Here's how the part is built. I have some questions about the finished solid (model axes, mm). Face numbers are marked on the shaded views. A direction names the side the tool comes from. Coordinates: 2 decimals unless noted, no trailing zeros. Write each loop counter-clockwise with the first axis right and the second up, starting at its lowest first coordinate (ties: lowest second). Pieces come first, ordered by that corner, then holes. Notation, with made-up numbers: (-17, 22) -> (42, 22) arc R29 ccw to (42, 57) -> close; hole circle Ø8 at (18.25, 87). An arc over 180 degrees is marked (long way). Use a Markdown table: item, result. Add a question column.
```python
from build123d import *

# Parameters (mm, degrees)
EXTRUDE1_DEPTH      = 7
EXTRUDE2_DEPTH      = 146.223964964
EXTRUDE2_DEPTH_BACK = 146.223964964
SKETCH2_R           = 2.6
SKETCH5_W           = 6
SKETCH5_H           = 3.7
EXTRUDE5_DEPTH      = 146.292807805
EXTRUDE6_DEPTH      = 3.7


with BuildPart() as part:
    # Sketch1 → Extrude1 (new, symmetric)
    with BuildSketch(Plane.XY):
        with BuildLine():
            Line((0, 0), (27.422252789, 0))
            ThreePointArc((27.422252789, 0), (27.989575353, 0.05413084), (28.536424818, 0.214569927))
            Line((28.536424818, 0.214569927), (37.105958636, 3.642383454))
            ThreePointArc((37.105958636, 3.642383454), (38.017374412, 3.909781934), (38.962912018, 4))
            Line((38.962912018, 4), (145, 4))
            Line((145, 4), (145, 2))
            Line((145, 2), (38.962912018, 2))
            ThreePointArc((38.962912018, 2), (38.395589454, 1.94586916), (37.848739989, 1.785430073))
            Line((37.848739989, 1.785430073), (29.279206171, -1.642383454))
            ThreePointArc((29.279206171, -1.642383454), (28.367790395, -1.909781934), (27.422252789, -2))
            Line((27.422252789, -2), (0, -2))
            Line((0, -2), (0, 0))
        make_face()
    extrude(amount=EXTRUDE1_DEPTH, both=True)

    # Sketch2 → Extrude2 (cut, two sides: drawn at the far end of the back side and taken through both)
    with BuildSketch(Plane(origin=(0, 0, 0), x_dir=(1, 0, 0), z_dir=(0, 1, 0)).offset(-EXTRUDE2_DEPTH_BACK)):
        with Locations(Location((8, 0, 0), (0, 0, 270))):
            Circle(SKETCH2_R)
        with Locations(Location((112, 0, 0), (0, 0, 270))):
            Circle(SKETCH2_R)
        with BuildLine():
            Line((138, 7), (138, 13.502314884))
            Line((138, 13.502314884), (156.33198023, 13.502314884))
            Line((156.33198023, 13.502314884), (156.33198023, -14.26269046))
            Line((156.33198023, -14.26269046), (138, -14.26269046))
            Line((138, -14.26269046), (138, -7))
            ThreePointArc((138, -7), (145, 0), (138, 7))
        make_face()
        with BuildLine():
            Line((7, 7), (7, 12.663603668))
            Line((7, 12.663603668), (-7.097085647, 12.663603668))
            Line((-7.097085647, 12.663603668), (-7.097085647, -11.053510543))
            Line((-7.097085647, -11.053510543), (7, -11.053510543))
            Line((7, -11.053510543), (7, -7))
            ThreePointArc((7, -7), (0, 0), (7, 7))
        make_face()
    extrude(amount=EXTRUDE2_DEPTH + EXTRUDE2_DEPTH_BACK, mode=Mode.SUBTRACT)

    # Sketch5 → Extrude5 (cut, through all)
    with BuildSketch(Plane(origin=(0, 4, 0), x_dir=(1, 0, 0), z_dir=(0, 1, 0))):
        with Locations((130, 5.15)):
            Rectangle(SKETCH5_W, SKETCH5_H)
    extrude(amount=-EXTRUDE5_DEPTH, mode=Mode.SUBTRACT)

    # Sketch6 → Extrude6 (add)
    with BuildSketch(Plane.XY.offset(-7)):
        with BuildLine():
            Line((125.978380641, 4), (124.313573726, 4))
            Line((124.313573726, 4), (124.313573726, 2))
            Line((124.313573726, 2), (126.730778484, 2))
            ThreePointArc((126.730778484, 2), (127.10118691, 2.071131011), (127.418900283, 2.274404804))
            ThreePointArc((127.418900283, 2.274404804), (129.995755169, 3.923082851), (133, 4.5))
            Line((133, 4.5), (133, 6.5))
            ThreePointArc((133, 6.5), (129.608718605, 5.914287154), (126.61035388, 4.22500979))
            ThreePointArc((126.61035388, 4.22500979), (126.313798135, 4.057930414), (125.978380641, 4))
        make_face()
    extrude(amount=EXTRUDE6_DEPTH)


solid = part.part
```
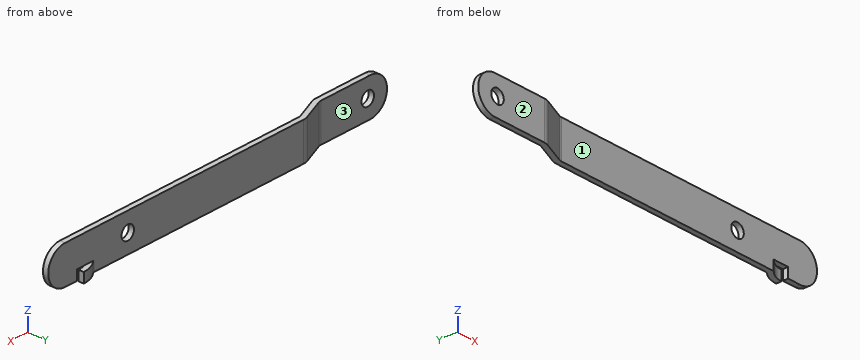
Q1. Suppose I cut it at D-D, the plane x = 80.5. Write out the boundary of the cut face in (y, z), and give its area (3 significant figures).
Q2. Suppose I cut it at C-C, the plane z = 5.5. Write out the boundary of the cut face in (x, y).
Q3. Suppose I cut it at B-B, the plane z = -0.5. Write out the boundary of the cut face in (x, y).
Q4. Will these pins go through, and if not, where does the flat tip stop? pin 1 (1 mm diameter, centred on y = 5.5, z = -5.5, fed in from +X); pin 2 (3 mm diameter, centred on y = 4.5, z = -5, fed in from +X); pin 3 (1.5 mm diameter, centred on y = -1, z = -2, fed in from -X).
Q5. Please list where these lines run through material, in increasing order: line 1 (Z direction, x = 112, y = 3.6); line 2 (Y direction, x = 124.5, z = 1); line 3 (Y direction, x = 21, z = -3.25).
Q6. Suppose I cut it at A-A, the plane x = 112. Write out the boundary of the cut face in (y, z).
Q7. Which directions (+Z, -Z, +X, -X, +Y, -Y) give clear straight access to the entire face, cutting with the end or side of a thin tool? Please do the marked faces 1, 2 and 3.
Answer key:
| question | item | result |
|---|---|---|
| 1 | outline | (2, -7) -> (4, -7) -> (4, 7) -> (2, 7) -> close |
| 1 | area | 28.0 mm^2 |
| 2 | outline | (2.67, -2) -> (27.42, -2) arc R5 ccw to (29.28, -1.64) -> (37.85, 1.79) arc R3 cw to (38.96, 2) -> (142.33, 2) -> (142.33, 4) -> (38.96, 4) arc R5 ccw to (37.11, 3.64) -> (28.54, 0.21) arc R3 cw to (27.42, 0) -> (2.67, 0) -> close |
| 3 | outline | (0.02, -2) -> (5.45, -2) -> (5.45, 0) -> (0.02, 0) -> close; (10.55, -2) -> (27.42, -2) arc R5 ccw to (29.28, -1.64) -> (37.85, 1.79) arc R3 cw to (38.96, 2) -> (109.45, 2) -> (109.45, 4) -> (38.96, 4) arc R5 ccw to (37.11, 3.64) -> (28.54, 0.21) arc R3 cw to (27.42, 0) -> (10.55, 0) -> close; (114.55, 2) -> (144.98, 2) -> (144.98, 4) -> (114.55, 4) -> close |
| 4 | pin 1 | stops at x = 133 |
| 4 | pin 2 | stops at x = 144.01 |
| 4 | pin 3 | stops at x = 0.11 |
| 5 | line 1 | z = -7 to -2.6, 2.6 to 7 |
| 5 | line 2 | y = 2 to 4 |
| 5 | line 3 | y = -2 to 0 |
| 6 | outline | (2, -7) -> (4, -7) -> (4, -2.6) -> (2, -2.6) -> close; (2, 2.6) -> (4, 2.6) -> (4, 7) -> (2, 7) -> close |
| 7 | face 1 | +Z, -Z, +X, -Y |
| 7 | face 2 | +Z, -Z, +X, -X, -Y |
| 7 | face 3 | +Z, -Z, -X, +Y |
